The drawing under review shows one solid part. Ordinate dimensions are in mm from its lowest x, y, z. A direction names the side the tool comes from. Round coordinates to 2 decimals unless told otherwise and drop trailing zeros. Loops run counter-clockwise (first coordinate to the right, second up) from the corner with the lowest first, then second, coordinate; pieces in that order, holes last. Notation, with made-up numbers: (17, 19.25) - (31, 19.25) arc R24 ccw to (31, 34.25) - close; hole circle Ø4 at (-27, 89). An arc over 180 degrees is marked (long way). Answer as CSV lines item,"result".
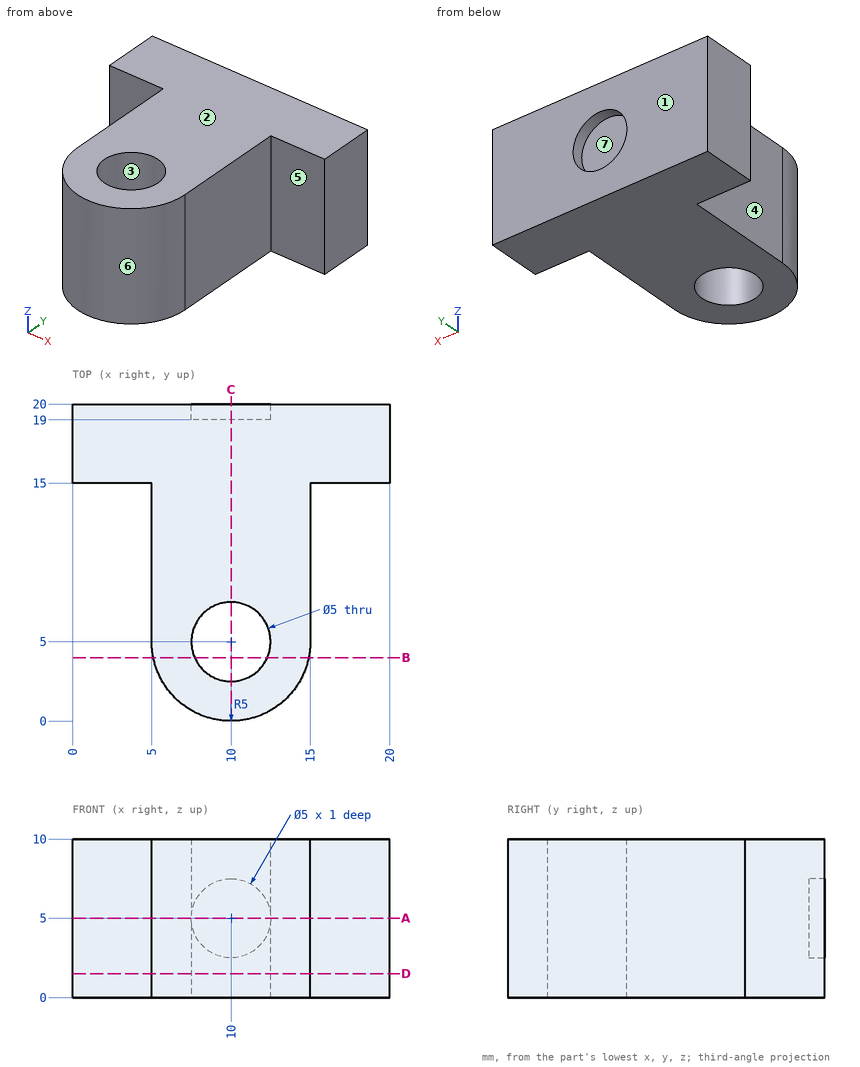
1. Draft analysis for pull direction Y (two halves, no side actions). For the marked faces 1, 2 and 3, state which applies: +Y half, -Y half, draft (parallel to the pull), parting line (faces both ways), or undercut.
Numbers:
face 1,"+Y half"
face 2,"draft"
face 3,"undercut"
2. Wall thickness on probe 1 along X at (y, z) = (19.7, 5); probe 2 along Y at (x, z) = (17.5, 8.75); probe 3 along X at (y, z) = (14, 4): over which ranges is each line inside the solid? List them lowest first.
Numbers:
probe 1,"x = 0 to 7.5, 12.5 to 20"
probe 2,"y = 15 to 20"
probe 3,"x = 5 to 15"
3. Take a section at D-D (z = 1.5). State the section outline as (x, y) points.
Numbers:
outline,"(0, 15) - (5, 15) - (5, 5) arc R5 ccw to (15, 5) - (15, 15) - (20, 15) - (20, 20) - (0, 20) - close; hole circle Ø5 at (10, 5)"
4. Take a section at C-C (x = 10). State the section outline as (y, z) points.
Numbers:
outline,"(0, 0) - (2.5, 0) - (2.5, 10) - (0, 10) - close; (7.5, 0) - (20, 0) - (20, 2.5) - (19, 2.5) - (19, 7.5) - (20, 7.5) - (20, 10) - (7.5, 10) - close"
5. Take a section at B-B (y = 4). State the section outline as (x, z) points.
Numbers:
outline,"(5.1, 0) - (7.71, 0) - (7.71, 10) - (5.1, 10) - close; (12.29, 0) - (14.9, 0) - (14.9, 10) - (12.29, 10) - close"
6. Clearance check with flat-ended pins moving along their axes: pin 1 (4 mm diameter, centred on x = 10, z = 6, fed in from +Y); pin 2 (6 mm diameter, centred on y = 6.5, z = 8.5, fed in from -X); pin 3 (5 mm diameter, centred on y = 10.5, z = 6, fed in from +X); pin 4 (1 mm diameter, centred on x = 3, z = 4, fed in from -Y). State where each tip first meets the part, or that it passes through.
Numbers:
pin 1,"stops at y = 20"
pin 2,"stops at x = 5"
pin 3,"stops at x = 15"
pin 4,"stops at y = 15"
7. Take a section at A-A (z = 5). State the section outline as (x, y) points, plus the area to 3 significant figures.
Numbers:
outline,"(0, 15) - (5, 15) - (5, 5) arc R5 ccw to (15, 5) - (15, 15) - (20, 15) - (20, 20) - (12.5, 20) - (12.5, 19) - (7.5, 19) - (7.5, 20) - (0, 20) - close; hole circle Ø5 at (10, 5)"
area,"215 mm²"
8. Tool access review of the marked faces 4, 5, 6 and 7: name each direction out of +Z, -Z, +X, -X, +Y, -Y from which nothing blocks a thin tool from reaching the whole face with its end or side.
Numbers:
face 4,"+Z, -Z, -X, -Y"
face 5,"+Z, -Z, +X, -Y"
face 6,"+Z, -Z, -Y"
face 7,"+Y"
